from build123d import *

# Parameters (mm, degrees)
FLANGE_PROFILE_R                 = 26
FLANGE_52_DEPTH                  = 5
HUB_PROFILE_R                    = 12.5
HUB_25_DEPTH                     = 7
BORE_16_DEPTH                    = 39.678159212
BORE_16_DEPTH_BACK               = 39.678159212
BORE_PROFILE_R                   = 8
BOLT_HOLES_3X_6_PCD35_DEPTH      = 38.429934544
BOLT_HOLES_3X_6_PCD35_DEPTH_BACK = 38.429934544
BOLT_HOLE_PROFILE_R              = 3
FLANGE_EDGE_FILLET_R2_R          = 2


with BuildPart() as part:
    # Flange Profile → Flange Ø52 (new body)
    with BuildSketch(Plane.XY):
        Circle(FLANGE_PROFILE_R)
    extrude(amount=-FLANGE_52_DEPTH)

    # Hub Profile → Hub Ø25 (add)
    with BuildSketch(Plane(origin=(0, 0, -5), x_dir=(-1, 0, 0), z_dir=(0, 0, -1))):
        Circle(HUB_PROFILE_R)
    extrude(amount=HUB_25_DEPTH)

    # Bore Profile → Bore Ø16 (cut, two sides: drawn at the far end of the back side and taken through both)
    with BuildSketch(Plane(origin=(0, 0, -12), x_dir=(-1, 0, 0), z_dir=(0, 0, -1)).offset(-BORE_16_DEPTH_BACK)):
        Circle(BORE_PROFILE_R)
    extrude(amount=BORE_16_DEPTH + BORE_16_DEPTH_BACK, mode=Mode.SUBTRACT)

    # Bolt Hole Profile → Bolt Holes 3xØ6 PCD35 (cut, two sides: drawn at the far end of the back side and taken through both)
    with BuildSketch(Plane(origin=(0, 0, -5), x_dir=(-1, 0, 0), z_dir=(0, 0, -1)).offset(-BOLT_HOLES_3X_6_PCD35_DEPTH_BACK)):
        with Locations((0, 17.5)):
            Circle(BOLT_HOLE_PROFILE_R)
        with Locations((15.155444566, -8.75)):
            Circle(BOLT_HOLE_PROFILE_R)
        with Locations((-15.155444566, -8.75)):
            Circle(BOLT_HOLE_PROFILE_R)
    extrude(amount=BOLT_HOLES_3X_6_PCD35_DEPTH + BOLT_HOLES_3X_6_PCD35_DEPTH_BACK, mode=Mode.SUBTRACT)

    # Flange Edge Fillet R2
    flange_edge_fillet_r2_edges = [part.edges().sort_by_distance(p)[0] for p in [
        (-26, 0, 0),
    ]]
    fillet(flange_edge_fillet_r2_edges, radius=FLANGE_EDGE_FILLET_R2_R)


solid = part.part
Build history of the part. All positions in model axes, mm. A direction names the side the tool comes from. Coordinates: 2 decimals unless noted, no trailing zeros. Write each loop counter-clockwise with the first axis right and the second up, starting at its lowest first coordinate (ties: lowest second). Pieces come first, ordered by that corner, then holes.
(1) Mould opens along Y. For faces 3 (the cylindrical face through (0.65, 14.57, -2.46)), 4 (the cylindrical face through (-11.923, 3.755, -8.451)), 5 (the flat face through (-6, 6, 0)) say: pulls with the +Y half, pulls with the -Y half, needs draft (parallel to the pull), parting line crosses it, or undercut.
(2) Cut at D-D on z = -9. List the corners of the cut face in (x, y).
(3) Cut at B-B on x = 0. List the corners of the cut face in (y, z).
(4) Cut at A-A on y = 0. List the corners of the cut face in (x, z), and give its area (3 significant figures).
(5) 3-axis set-ups, long thin cutter, end or side, ignore diameter. For faces 1 (the flat face through (0.2, -8.2, -12)), 2 (the flat face through (-6.1, -11.2, -5)): which of +Z, -Z, +X, -X, +Y, -Y reach the whole face in a straight line?
(6) Drill centre lines: line 1 (X direction, y = -8.75, z = -3.5); line 2 (X direction, y = -8.75, z = -1.1); line 3 (Y direction, x = 2.5, z = -3). Where is each one in solid material? Low to high.
(7) Pin check, flat tips, straight feed: pin 1 Ø5.5 at (x, y) = (-15.16, -8.75) entering from -Z; pin 2 Ø1.5 at (x, y) = (11.5, -14) entering from -Z; pin 3 Ø4 at (x, z) = (-7, -7.5) entering from -Y; pin 4 Ø4 at (y, z) = (3, -1.5) entering from +X. Stop position of each tip, or through.
(8) Cut at C-C on z = -4. List the corners of the cut face in (x, y).
Working result:
1. face 3: undercut
1. face 4: parting line crosses it
1. face 5: needs draft
2. outline: circle Ø25 at (0, 0); hole circle Ø16 at (0, 0)
3. outline: (-26, -5) - (-12.5, -5) - (-12.5, -12) - (-8, -12) - (-8, 0) - (-24, 0) arc R2 ccw to (-26, -2) - close; (8, -12) - (12.5, -12) - (12.5, -5) - (14.5, -5) - (14.5, 0) - (8, 0) - close; (20.5, -5) - (26, -5) - (26, -2) arc R2 ccw to (24, 0) - (20.5, 0) - close
4. outline: (-26, -5) - (-12.5, -5) - (-12.5, -12) - (-8, -12) - (-8, 0) - (-24, 0) arc R2 ccw to (-26, -2) - close; (8, -12) - (12.5, -12) - (12.5, -5) - (26, -5) - (26, -2) arc R2 ccw to (24, 0) - (8, 0) - close
4. area: 241 mm2
5. face 1: -Z, +X, -X, +Y, -Y
5. face 2: -Z
6. line 1: x = -24.48 to -18.16, -12.16 to 12.16, 18.16 to 24.48
6. line 2: x = -24.26 to -18.16, -12.16 to 12.16, 18.16 to 24.26
6. line 3: y = -25.88 to -7.6, 7.6 to 15.84, 19.16 to 25.88
7. pin 1: passes through
7. pin 2: stops at z = -5
7. pin 3: stops at y = -11.46
7. pin 4: stops at x = 25.98
8. outline: circle Ø52 at (0, 0); hole circle Ø6 at (-15.16, -8.75); hole circle Ø16 at (0, 0); hole circle Ø6 at (0, 17.5); hole circle Ø6 at (15.16, -8.75)
